from build123d import *

# Parameters (mm, degrees)
EXTRUDE1_DEPTH             = 10
SKETCH2_OUTSIDE_W          = 30.536
SKETCH2_OUTSIDE_H          = 30.536
SKETCH2_OUTSIDE_R          = 9
EXTRUDE2_DEPTH             = 1
M4X0_7_TAPPED_HOLE1_D      = 3.3
M4X0_7_TAPPED_HOLE1_DEPTH  = 10.1
M4X0_7_TAPPED_HOLE1_TIP    = 0.991420021
M12X1_5_TAPPED_HOLE1_D     = 10.5
M12X1_5_TAPPED_HOLE1_DEPTH = 28.5
M12X1_5_TAPPED_HOLE1_TIP   = 3.15451825


with BuildPart() as part:
    # Sketch1 → Extrude1 (new body)
    with BuildSketch(Plane.XY):
        with BuildLine():
            Line((-5.937171043, -11), (5.937171043, -11))
            ThreePointArc((5.937171043, -11), (8.838834765, -8.838834765), (11, -5.937171043))
            Line((11, -5.937171043), (11, 5.937171043))
            ThreePointArc((11, 5.937171043), (8.838834765, 8.838834765), (5.937171043, 11))
            Line((5.937171043, 11), (-5.937171043, 11))
            ThreePointArc((-5.937171043, 11), (-8.838834765, 8.838834765), (-11, 5.937171043))
            Line((-11, 5.937171043), (-11, -5.937171043))
            ThreePointArc((-11, -5.937171043), (-8.838834765, -8.838834765), (-5.937171043, -11))
        make_face()
    extrude(amount=EXTRUDE1_DEPTH)

    # Sketch2 outside → Extrude2 (cut)
    with BuildSketch(Plane.XY.offset(10)):
        Rectangle(SKETCH2_OUTSIDE_W, SKETCH2_OUTSIDE_H)
        Circle(SKETCH2_OUTSIDE_R, mode=Mode.SUBTRACT)
    extrude(amount=-EXTRUDE2_DEPTH, mode=Mode.SUBTRACT)

    # M4x0.7 Tapped Hole1
    with Locations(Plane(origin=(-8.535457879, 9.132138785, 4.649594026), x_dir=(0.730571102805, 0.682836630349, 0), z_dir=(-0.682836630349, 0.730571102805, 0))):
        with Locations((0, 0)):
            Hole(M4X0_7_TAPPED_HOLE1_D / 2, depth=M4X0_7_TAPPED_HOLE1_DEPTH)
            with Locations((0, 0, -(M4X0_7_TAPPED_HOLE1_DEPTH + M4X0_7_TAPPED_HOLE1_TIP / 2))):  # 118° drill point
                Cone(0, M4X0_7_TAPPED_HOLE1_D / 2, M4X0_7_TAPPED_HOLE1_TIP, mode=Mode.SUBTRACT)

    # M12x1.5 Tapped Hole1
    with Locations(Plane.XY.offset(10)):
        with Locations((0, 0)):
            Hole(M12X1_5_TAPPED_HOLE1_D / 2, depth=M12X1_5_TAPPED_HOLE1_DEPTH)
            with Locations((0, 0, -(M12X1_5_TAPPED_HOLE1_DEPTH + M12X1_5_TAPPED_HOLE1_TIP / 2))):  # 118° drill point
                Cone(0, M12X1_5_TAPPED_HOLE1_D / 2, M12X1_5_TAPPED_HOLE1_TIP, mode=Mode.SUBTRACT)


solid = part.part
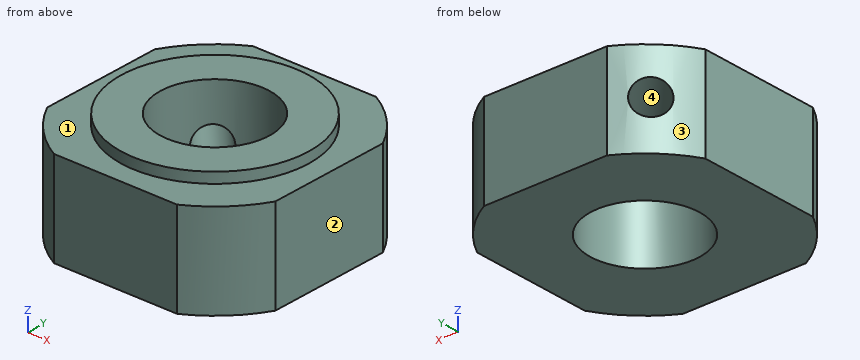
Geometry: final body of the model. Coordinates: model frame, mm. Face numbers are marked on the shaded views. Coordinates: 2 decimals unless noted, no trailing zeros. Write each loop counter-clockwise with the first axis right and the second up, starting at its lowest first coordinate (ties: lowest second). Pieces come first, ordered by that corner, then holes. Notation, with made-up numbers: (49.5, 7) - (86.5, 7) arc R8 ccw to (86.5, 15) - close; hole circle Ø6 at (-23.75, -27). An arc over 180 degrees is marked (long way). Return JSON: item names as keys, results as strings.
Item 1: Section query C-C (z = 5). Output: boundary loops of the cut face in (x, y), and give its area (3 significant figures).
Completed:
{"outline": "(-11, -5.94) arc R12.5 ccw to (-5.94, -11) - (5.94, -11) arc R12.5 ccw to (11, -5.94) - (11, 5.94) arc R12.5 ccw to (5.94, 11) - (-5.94, 11) arc R12.5 ccw to (-7.29, 10.16) - (-2.23, 4.75) arc R5.25 cw (long way) to (-4.59, 2.55) - (-9.64, 7.95) arc R12.5 ccw to (-11, 5.94) - close", "area": "333 mm2"}
Item 2: Section query D-D (y = -7). Output: boundary loops of the cut face in (x, z).
Completed:
{"outline": "(-10.36, 0) - (10.36, 0) - (10.36, 9) - (5.66, 9) - (5.66, 10) - (-5.66, 10) - (-5.66, 9) - (-10.36, 9) - close"}
Item 3: Pull-direction query (X, two-part tool) for the marked faces 1, 2, 3 and 4; classes: +X half, -X half, draft (parallel to the pull), parting line (faces both ways), or undercut.
Completed:
{"face 1": "draft", "face 2": "+X half", "face 3": "-X half", "face 4": "undercut"}
Item 4: Pin query (flat end, axial travel): pin 1 Ø4 at (y, z) = (-8, 4) entering from +X; pin 2 Ø4 at (x, z) = (-9, 8.5) entering from -Y. Return the tip coordinate at first contact, or that it passes through.
Completed:
{"pin 1": "stops at x = 10.97", "pin 2": "stops at y = -10.36"}
Item 5: Line query: L1, parallel to Y at x = 0, z = 4.5; L2, parallel to Z at x = -9.5, y = 2.75; L3, parallel to X at y = -0.5, z = 0.75. Output: solid intervals per line, ascending.
Completed:
{"L1": "y = -11 to -5.25, 5.25 to 11", "L2": "z = 0 to 9", "L3": "x = -11 to -5.23, 5.23 to 11"}
Item 6: Section query A-A (y = 0). Output: boundary loops of the cut face in (x, z).
Completed:
{"outline": "(-11, 0) - (-5.25, 0) - (-5.25, 10) - (-9, 10) - (-9, 9) - (-11, 9) - close; (5.25, 0) - (11, 0) - (11, 9) - (9, 9) - (9, 10) - (5.25, 10) - close"}
